CAD build for the part. Positions are in the model's coordinates, mm. A direction names the side the tool comes from. Round coordinates to 2 decimals unless told otherwise and drop trailing zeros. Loops run counter-clockwise (first coordinate to the right, second up) from the corner with the lowest first, then second, coordinate; pieces in that order, holes last. Notation, with made-up numbers: M 10.5,23 L 19.5,23 A21 cw 19.5,32 Z; hole C 71,-12.75 d5. An arc over 180 degrees is marked long. Use one line per item in the form item = value.
from build123d import *

# Parameters (mm, degrees)
BOSS_EXTRUDE2_DEPTH = 20
SKETCH4_W           = 10.5
SKETCH4_H           = 6
BOSS_EXTRUDE3_DEPTH = 20


with BuildPart() as part:
    # Sketch3 → Boss-Extrude2 (new, symmetric)
    with BuildSketch(Plane.XY):
        Polygon((0, 0), (10.5, 0), (37.498965991, -34.995654522), (42.249507329, -31.330636514), (13.449114839, 6), (0, 6), align=None)
    extrude(amount=BOSS_EXTRUDE2_DEPTH, both=True)

    # Sketch4 → Boss-Extrude3 (add)
    with BuildSketch(Plane.XY.offset(20)):
        with Locations((5.25, 3)):
            Rectangle(SKETCH4_W, SKETCH4_H)
    boss_extrude3 = extrude(amount=BOSS_EXTRUDE3_DEPTH)

    # Mirror1: Boss-Extrude3 across plane
    add(boss_extrude3.mirror(Plane.XY))


solid = part.part
1. Cut at B-B on y = 1. Write the cut outline in (x, z).
Completed:
outline = M 0,-40 L 10.5,-40 L 10.5,-20 L 17.31,-20 L 17.31,20 L 10.5,20 L 10.5,40 L 0,40 Z
2. Cut at D-D on z = 33. Write the cut outline in (x, y).
Completed:
outline = M 0,0 L 10.5,0 L 10.5,6 L 0,6 Z
3. Drop flat-ended pins along their axis: P1, Ø3, axis at y = -20, z = 8.5, coming from the +X side; P2, Ø12, axis at x = 21, y = -1.5, coming from the +Z side; P3, Ø3, axis at y = 1.5, z = -30.5, coming from the +X side. Give the stop position or say it passes through.
Completed:
P1 = 34.67
P2 = 20
P3 = 10.5
4. Cut at A-A on z = -18. Write the cut outline in (x, y), and give its area (3 significant figures).
Completed:
outline = M 0,0 L 10.5,0 L 37.5,-35 L 42.25,-31.33 L 13.45,6 L 0,6 Z
area = 346 mm2
5. Cut at C-C on x = 8.5. Write the cut outline in (y, z), and give its area (3 significant figures).
Completed:
outline = M 0,-40 L 6,-40 L 6,40 L 0,40 Z
area = 480 mm2
6. Probe line 1 along Z through (x, y) = (25, -11.5); line 2 along X through (y, z) = (-32.5, 17); line 3 along Y through (x, z) = (8, 18). List the from-to ranges inside material, lowest first. Write a range as from..to.
Completed:
line_1 = -20..20
line_2 = 35.57..40.73
line_3 = 0..6
7. Tool access for faces 1 (the face through (10.5, 3, -30)), 2 (the face through (39.84, -33.19, 0.28)), 3 (the face through (10.5, 3, 30)), 4 (the face through (5, 0, 1)): list every direction of +Z, -Z, +X, -X, +Y, -Y with a clear straight run to the whole face (end or side of a thin tool).
Completed:
face_1 = -Z, +X, +Y, -Y
face_2 = +Z, -Z, +X, -Y
face_3 = +Z, +X, +Y, -Y
face_4 = +Z, -Z, -X, -Y
